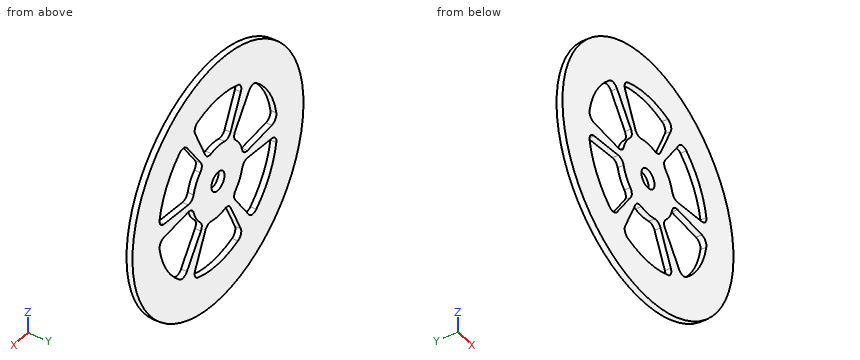
from build123d import *

# Parameters (mm, degrees)
SKETCH1_R           = 85
SKETCH1_R_2         = 6.5
BOSS_EXTRUDE1_DEPTH = 4
CUT_EXTRUDE1_DEPTH  = 10
FILLET1_R           = 5


with BuildPart() as part:
    # Sketch1 → Boss-Extrude1 (new body)
    with BuildSketch(Plane(origin=(0, 0, 0), x_dir=(1, 0, 0), z_dir=(0, 1, 0))):
        with Locations(Location((0, 0, 0), (0, 0, 270))):
            Circle(SKETCH1_R)
        with Locations(Location((0, 0, 0), (0, 0, 270))):
            Circle(SKETCH1_R_2, mode=Mode.SUBTRACT)
    extrude(amount=BOSS_EXTRUDE1_DEPTH)

    # Sketch2 → Cut-Extrude1 (cut)
    with BuildSketch(Plane(origin=(0, 4, 0), x_dir=(1, 0, 0), z_dir=(0, 1, 0))):
        with BuildLine():
            Line((10.565456544, 22.657694676), (24.934477443, 53.472159435))
            ThreePointArc((24.934477443, 53.472159435), (0, 59), (-24.934477443, 53.472159435))
            Line((-24.934477443, 53.472159435), (-10.565456544, 22.657694676))
            ThreePointArc((-10.565456544, 22.657694676), (0, 25), (10.565456544, 22.657694676))
        make_face()
        with BuildLine():
            Line((14.339410909, 20.478801107), (33.841009745, 48.329970613))
            ThreePointArc((33.841009745, 48.329970613), (51.095498823, 29.5), (58.775487187, 5.142188822))
            Line((58.775487187, 5.142188822), (24.904867452, 2.178893569))
            ThreePointArc((24.904867452, 2.178893569), (21.650635095, 12.5), (14.339410909, 20.478801107))
        make_face()
        with BuildLine():
            Line((24.904867452, -2.178893569), (58.775487187, -5.142188822))
            ThreePointArc((58.775487187, -5.142188822), (51.095498823, -29.5), (33.841009745, -48.329970613))
            Line((33.841009745, -48.329970613), (14.339410909, -20.478801107))
            ThreePointArc((14.339410909, -20.478801107), (21.650635095, -12.5), (24.904867452, -2.178893569))
        make_face()
        with BuildLine():
            Line((10.565456544, -22.657694676), (24.934477443, -53.472159435))
            ThreePointArc((24.934477443, -53.472159435), (0, -59), (-24.934477443, -53.472159435))
            Line((-24.934477443, -53.472159435), (-10.565456544, -22.657694676))
            ThreePointArc((-10.565456544, -22.657694676), (0, -25), (10.565456544, -22.657694676))
        make_face()
        with BuildLine():
            Line((-14.339410909, -20.478801107), (-33.841009745, -48.329970613))
            ThreePointArc((-33.841009745, -48.329970613), (-51.095498823, -29.5), (-58.775487187, -5.142188822))
            Line((-58.775487187, -5.142188822), (-24.904867452, -2.178893569))
            ThreePointArc((-24.904867452, -2.178893569), (-21.650635095, -12.5), (-14.339410909, -20.478801107))
        make_face()
        with BuildLine():
            Line((-24.904867452, 2.178893569), (-58.775487187, 5.142188822))
            ThreePointArc((-58.775487187, 5.142188822), (-51.095498823, 29.5), (-33.841009745, 48.329970613))
            Line((-33.841009745, 48.329970613), (-14.339410909, 20.478801107))
            ThreePointArc((-14.339410909, 20.478801107), (-21.650635095, 12.5), (-24.904867452, 2.178893569))
        make_face()
    extrude(amount=-CUT_EXTRUDE1_DEPTH, mode=Mode.SUBTRACT)

    # Fillet1
    fillet1_edges = [part.edges().sort_by_distance(p)[0] for p in [
        (-10.565456544, 2, 22.657694676),
        (10.565456544, 2, 22.657694676),
        (24.934477443, 2, 53.472159435),
        (-24.934477443, 2, 53.472159435),
        (-24.904867452, 2, 2.178893569),
        (-14.339410909, 2, 20.478801107),
        (-33.841009745, 2, 48.329970613),
        (-58.775487187, 2, 5.142188822),
        (14.339410909, 2, 20.478801107),
        (24.904867452, 2, 2.178893569),
        (58.775487187, 2, 5.142188822),
        (33.841009745, 2, 48.329970613),
        (24.904867452, 2, -2.178893569),
        (14.339410909, 2, -20.478801107),
        (33.841009745, 2, -48.329970613),
        (58.775487187, 2, -5.142188822),
        (-14.339410909, 2, -20.478801107),
        (-24.904867452, 2, -2.178893569),
        (-58.775487187, 2, -5.142188822),
        (-33.841009745, 2, -48.329970613),
        (10.565456544, 2, -22.657694676),
        (-10.565456544, 2, -22.657694676),
        (-24.934477443, 2, -53.472159435),
        (24.934477443, 2, -53.472159435),
    ]]
    fillet(fillet1_edges, radius=FILLET1_R)


solid = part.part
Source: CAD feature listing. Evaluate the final solid. Frame: model axes, mm. Give positions to 0.01 mm unless a question says otherwise; leave off trailing zeros. Write each loop counter-clockwise with the first axis right and the second up, starting at its lowest first coordinate (ties: lowest second). Pieces come first, ordered by that corner, then holes. Notation, with made-up numbers: (2, 78) -> (21, 78) arc R25 cw to (21, 107) -> close; hole circle Ø10 at (-5, 29.5). An arc over 180 degrees is marked (long way). Return JSON: item names as keys, results as strings. Group by question number.
1. Material intervals for line 1 (X direction, y = 2.05, z = 0); line 2 (X direction, y = 1.5, z = 15.5); line 3 (X direction, y = 1.2, z = 14), sorted ascending. Write a range as from..to.
2. Section B-B, the plane z = 0. Output: boundary loops of the cut face in (x, y), then the cut area to 3 significant figures.
3. Section C-C, the plane z = -41. Output: boundary loops of the cut face in (x, y), then the cut area to 3 significant figures.
4. Section D-D, the plane x = -51. Output: boundary loops of the cut face in (y, z).
5. Section A-A, the plane x = 0. Output: boundary loops of the cut face in (y, z).
6. Pin query (flat end, axial travel): pin 1 Ø1.5 at (y, z) = (3, 67.5) entering from -X; pin 2 Ø1.5 at (x, z) = (-11, -55.5) entering from -Y. Return the tip coordinate at first contact, or that it passes through.
Determined:
{
 "1": {"line 1": "x = -85..-6.5, 6.5..85", "line 2": "x = -83.57..-56.93, -19.62..19.62, 56.93..83.57", "line 3": "x = -83.84..-57.31, -20.71..20.71, 57.31..83.84"},
 "2": {"outline": "(-85, 0) -> (-6.5, 0) -> (-6.5, 4) -> (-85, 4) -> close; (6.5, 0) -> (85, 0) -> (85, 4) -> (6.5, 4) -> close", "area": "628 mm2"},
 "3": {"outline": "(-74.46, 0) -> (-42.43, 0) -> (-42.43, 4) -> (-74.46, 4) -> close; (-28.71, 0) -> (-19.12, 0) -> (-19.12, 4) -> (-28.71, 4) -> close; (19.12, 0) -> (28.71, 0) -> (28.71, 4) -> (19.12, 4) -> close; (42.43, 0) -> (74.46, 0) -> (74.46, 4) -> (42.43, 4) -> close", "area": "333 mm2"},
 "4": {"outline": "(0, -68) -> (4, -68) -> (4, -29.66) -> (0, -29.66) -> close; (0, -4.46) -> (4, -4.46) -> (4, 4.46) -> (0, 4.46) -> close; (0, 29.66) -> (4, 29.66) -> (4, 68) -> (0, 68) -> close"},
 "5": {"outline": "(0, -85) -> (4, -85) -> (4, -59) -> (0, -59) -> close; (0, -25) -> (4, -25) -> (4, -6.5) -> (0, -6.5) -> close; (0, 6.5) -> (4, 6.5) -> (4, 25) -> (0, 25) -> close; (0, 59) -> (4, 59) -> (4, 85) -> (0, 85) -> close"},
 "6": {"pin 1": "stops at x = -52.63", "pin 2": "passes through"}
}
